from build123d import *

# Parameters (mm, degrees)
SKETCH1_R           = 10
BOSS_EXTRUDE1_DEPTH = 340
SKETCH2_OUTSIDE_W   = 90.234
SKETCH2_OUTSIDE_H   = 90.234
SKETCH2_OUTSIDE_W_2 = 12
SKETCH2_OUTSIDE_H_2 = 12
CUT_EXTRUDE1_DEPTH  = 27
SKETCH3_R           = 15
BOSS_EXTRUDE2_DEPTH = 8


with BuildPart() as part:
    # Sketch1 → Boss-Extrude1 (new body)
    with BuildSketch(Plane(origin=(0, 0, 0), x_dir=(1, 0, 0), z_dir=(0, 1, 0))):
        with Locations(Location((0, 0, 0), (0, 0, 270))):
            Circle(SKETCH1_R)
    extrude(amount=BOSS_EXTRUDE1_DEPTH)

    # Sketch2 outside → Cut-Extrude1 (cut)
    with BuildSketch(Plane(origin=(0, 340, 0), x_dir=(1, 0, 0), z_dir=(0, 1, 0))):
        Rectangle(SKETCH2_OUTSIDE_W, SKETCH2_OUTSIDE_H)
        Rectangle(SKETCH2_OUTSIDE_W_2, SKETCH2_OUTSIDE_H_2, mode=Mode.SUBTRACT)
    extrude(amount=-CUT_EXTRUDE1_DEPTH, mode=Mode.SUBTRACT)

    # Sketch3 → Boss-Extrude2 (add)
    with BuildSketch(Plane(origin=(0, 282, 0), x_dir=(1, 0, 0), z_dir=(0, 1, 0))):
        with Locations(Location((0, 0, 0), (0, 0, 270))):
            Circle(SKETCH3_R)
    extrude(amount=BOSS_EXTRUDE2_DEPTH)


solid = part.part
Can you work these out from the model? Positions are in its coordinate system, mm. A direction names the side the tool comes from. Coordinates: 2 decimals unless noted, no trailing zeros. Order: outer loops, then holes, each group sorted by start corner. A loop starts at its lowest first (then second) coordinate and runs counter-clockwise, first axis right, second up. Notation, with made-up numbers: M -5.75,-5 L 30.25,-5 A29 ccw 30.25,16 Z; hole C 23,-26 d3. An arc over 180 degrees is marked long. Answer as CSV lines item,"result".
(1) Suppose I cut it at B-B on x = 0. Please give me the cut outline in (y, z).
Geometry check:
outline,"M 0,-10 L 282,-10 L 282,-15 L 290,-15 L 290,-10 L 313,-10 L 313,-6 L 340,-6 L 340,6 L 313,6 L 313,10 L 290,10 L 290,15 L 282,15 L 282,10 L 0,10 Z"
(2) I'm going to push flat-ended pins straight in: pin 1 (1 mm diameter, centred on y = 158, z = 1, fed in from +X); pin 2 (8 mm diameter, centred on x = -4.5, y = 172.5, fed in from -Z); pin 3 (5 mm diameter, centred on y = 246.5, z = -7, fed in from -X). Where does each tip first touch, or does it pass through?
Geometry check:
pin 1,"x = 9.99"
pin 2,"z = -9.99"
pin 3,"x = -8.93"
(3) Suppose I cut it at A-A on z = 0. Please give me the cut outline in (x, y), plus the area to 3 significant figures.
Geometry check:
outline,"M -15,282 L -10,282 L -10,0 L 10,0 L 10,282 L 15,282 L 15,290 L 10,290 L 10,313 L 6,313 L 6,340 L -6,340 L -6,313 L -10,313 L -10,290 L -15,290 Z"
area,"6,660 mm^2"
(4) Suppose I cut it at C-C on y = 266.5. Please give me the cut outline in (x, z), plus the area to 3 significant figures.
Geometry check:
outline,"C 0,0 d20"
area,"314 mm^2"
(5) Please list where these lines run through material, in increasing order: L1, parallel to Y at x = -13.25, z = -4; L2, parallel to Z at x = 0, y = 130.5; L3, parallel to X at y = 213, z = 0.75.
Geometry check:
L1,"282 to 290"
L2,"-10 to 10"
L3,"-9.97 to 9.97"
(6) On a 3-axis mill with a long thin cutter (end or side, diameter ignored), from which of +Z, -Z, +X, -X, +Y, -Y can I reach the whole of each face in a straight line? I mean faces 1 (the flat face through (-10, 282, 3)), 2 (the flat face through (0, 327, -6)), 3 (the flat face through (0, 327, 6)), 4 (the flat face through (-6, 327, 0)), 5 (the cylindrical face through (-9.76, 301.34, -2.17)). Say none if no direction works.
Geometry check:
face 1,"-Y"
face 2,"-Z, +X, -X, +Y"
face 3,"+Z, +X, -X, +Y"
face 4,"+Z, -Z, -X, +Y"
face 5,"+Y"
